Check sheet for the modelled part. Datum: model origin and axes. Units: mm. Face numbers are marked on the shaded views. A direction names the side the tool comes from. Give positions to 0.01 mm unless a question says otherwise; leave off trailing zeros. Order: outer loops, then holes, each group sorted by start corner. A loop starts at its lowest first (then second) coordinate and runs counter-clockwise, first axis right, second up. Notation, with made-up numbers: (5, 52.25) - (43, 52.25) arc R23 ccw to (43, 67.25) - close; hole circle Ø7 at (78.5, 1). An arc over 180 degrees is marked (long way). Answer in a Markdown table with one row per item.
from build123d import *

# Parameters (mm, degrees)
EXTRUDE_1_DEPTH     = 10
SKETCH_2_R          = 2.1
CUT_EXTRUDE_1_DEPTH = 17.7


with BuildPart() as part:
    # 草图1 → 凸台-拉伸1 (new body)
    with BuildSketch(Plane.XY):
        with BuildLine():
            Line((-5.596661991, 5.185089456), (-5.596661991, 6.985089456))
            ThreePointArc((-5.596661991, 6.985089456), (0.053338009, 12.635089456), (5.703338009, 6.985089456))
            Line((5.703338009, 6.985089456), (5.703338009, 5.185089456))
            Line((5.703338009, 5.185089456), (5.703338009, 1.335089456))
            Line((5.703338009, 1.335089456), (15.053338009, 1.335089456))
            Line((15.053338009, 1.335089456), (15.053338009, 5.185089456))
            Line((15.053338009, 5.185089456), (8.65, 5.185089456))
            Line((8.65, 5.185089456), (8.65, 6.985089456))
            ThreePointArc((8.65, 6.985089456), (0, 15.635089456), (-8.65, 6.985089456))
            Line((-8.65, 6.985089456), (-8.65, 5.185089456))
            Line((-8.65, 5.185089456), (-14.946661991, 5.185089456))
            Line((-14.946661991, 5.185089456), (-14.946661991, 1.335089456))
            Line((-14.946661991, 1.335089456), (-5.596661991, 1.335089456))
            Line((-5.596661991, 1.335089456), (-5.596661991, 5.185089456))
        make_face()
    extrude(amount=EXTRUDE_1_DEPTH)

    # 草图2 → 切除-拉伸1 (cut)
    with BuildSketch(Plane(origin=(-970.090594905, 5.185089456, 1019.250263045), x_dir=(0, 0, 1), z_dir=(0, 1, 0))):
        with Locations((-1055.250263055, 981.942263912)):
            Circle(SKETCH_2_R)
        with Locations((-1055.250263055, 958.292263912)):
            Circle(SKETCH_2_R)
        with Locations((-1014.250263055, 958.292263912)):
            Circle(SKETCH_2_R)
        with Locations((-1014.250263055, 981.942263912)):
            Circle(SKETCH_2_R)
    extrude(amount=-CUT_EXTRUDE_1_DEPTH, mode=Mode.SUBTRACT)


solid = part.part
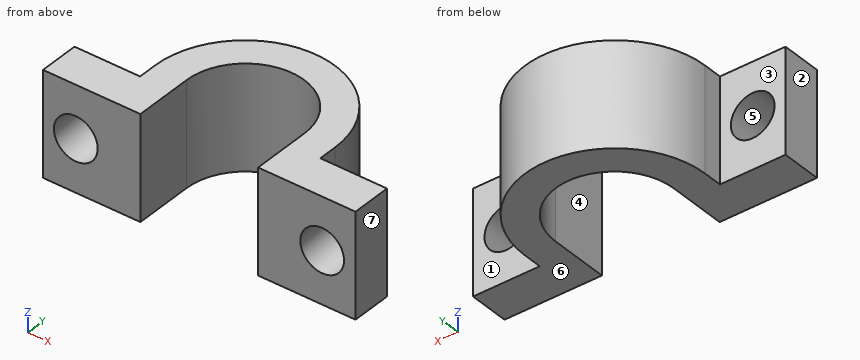
(1) Gauge pin test, flat ends, axial feed: P1, Ø3, axis at x = 13, z = 6, coming from the +Y side; P2, Ø0.5, axis at y = 6, z = 3, coming from the +X side; P3, Ø1.5, axis at y = 11, z = 4, coming from the +X side; P4, Ø5, axis at x = 9, y = 7, coming from the +Z side. Record the tip position at first contact, or that the pin passes through.
Geometry says:
| item | result |
|---|---|
| P1 | y = 5.19 |
| P2 | x = 8.65 |
| P3 | x = 8.01 |
| P4 | z = 10 |
(2) Mould release check, pull along X, two halves, no side actions. Record for the marked faces 5, 6 and 7: pulls with the +X half, pulls with the -X half, needs draft (parallel to the pull), parting line crosses it, or undercut.
Geometry says:
| item | result |
|---|---|
| face 5 | undercut |
| face 6 | needs draft |
| face 7 | pulls with the +X half |
(3) Cross-section at C-C, the plane x = 13. Record the cut outline in (y, z).
Geometry says:
| item | result |
|---|---|
| outline | (1.34, 0) - (5.19, 0) - (5.19, 3.24) - (1.34, 3.24) - close; (1.34, 6.76) - (5.19, 6.76) - (5.19, 10) - (1.34, 10) - close |
(4) Cross-section at D-D, the plane z = 8.5. Record the cut outline in (x, y).
Geometry says:
| item | result |
|---|---|
| outline | (-14.95, 1.34) - (-5.6, 1.34) - (-5.6, 6.99) arc R5.65 cw to (5.7, 6.99) - (5.7, 1.34) - (15.05, 1.34) - (15.05, 5.19) - (8.65, 5.19) - (8.65, 6.99) arc R8.65 ccw to (-8.65, 6.99) - (-8.65, 5.19) - (-14.95, 5.19) - close |
(5) Thickness scan on L1, parallel to X at y = 3.55, z = 5; L2, parallel to X at y = 4.25, z = 4.75; L3, parallel to X at y = 4.75, z = 1.5. Record the ranges inside material, lowest first.
Geometry says:
| item | result |
|---|---|
| L1 | -14.95 to -13.9, -9.7 to -5.6, 5.7 to 9.75, 13.95 to 15.05 |
| L2 | -14.95 to -13.88, -9.71 to -5.6, 5.7 to 9.77, 13.94 to 15.05 |
| L3 | -14.95 to -5.6, 5.7 to 15.05 |
(6) Cross-section at B-B, the plane y = 10. Record the cut outline in (x, z), then the cut area to 3 significant figures.
Geometry says:
| item | result |
|---|---|
| outline | (-8.11, 0) - (-4.73, 0) - (-4.73, 10) - (-8.11, 10) - close; (4.83, 0) - (8.11, 0) - (8.11, 10) - (4.83, 10) - close |
| area | 66.6 mm² |
(7) Cross-section at A-A, the plane z = 5. Record the cut outline in (x, y), then the cut area to 3 significant figures.
Geometry says:
| item | result |
|---|---|
| outline | (-14.95, 1.34) - (-13.9, 1.34) - (-13.9, 5.19) - (-14.95, 5.19) - close; (-9.7, 1.34) - (-5.6, 1.34) - (-5.6, 6.99) arc R5.65 cw to (5.7, 6.99) - (5.7, 1.34) - (9.75, 1.34) - (9.75, 5.19) - (8.65, 5.19) - (8.65, 6.99) arc R8.65 ccw to (-8.65, 6.99) - (-8.65, 5.19) - (-9.7, 5.19) - close; (13.95, 1.34) - (15.05, 1.34) - (15.05, 5.19) - (13.95, 5.19) - close |
| area | 118 mm² |
(8) Access from +Z, -Z, +X, -X, +Y, -Y to the whole of each face (thin tool, end or side, straight path). Record for the marked faces 1, 2, 3 and 4.
Geometry says:
| item | result |
|---|---|
| face 1 | +Z, -Z, +X, +Y |
| face 2 | +Z, -Z, -X, +Y, -Y |
| face 3 | +Z, -Z, -X, +Y |
| face 4 | +Z, -Z, -Y |
